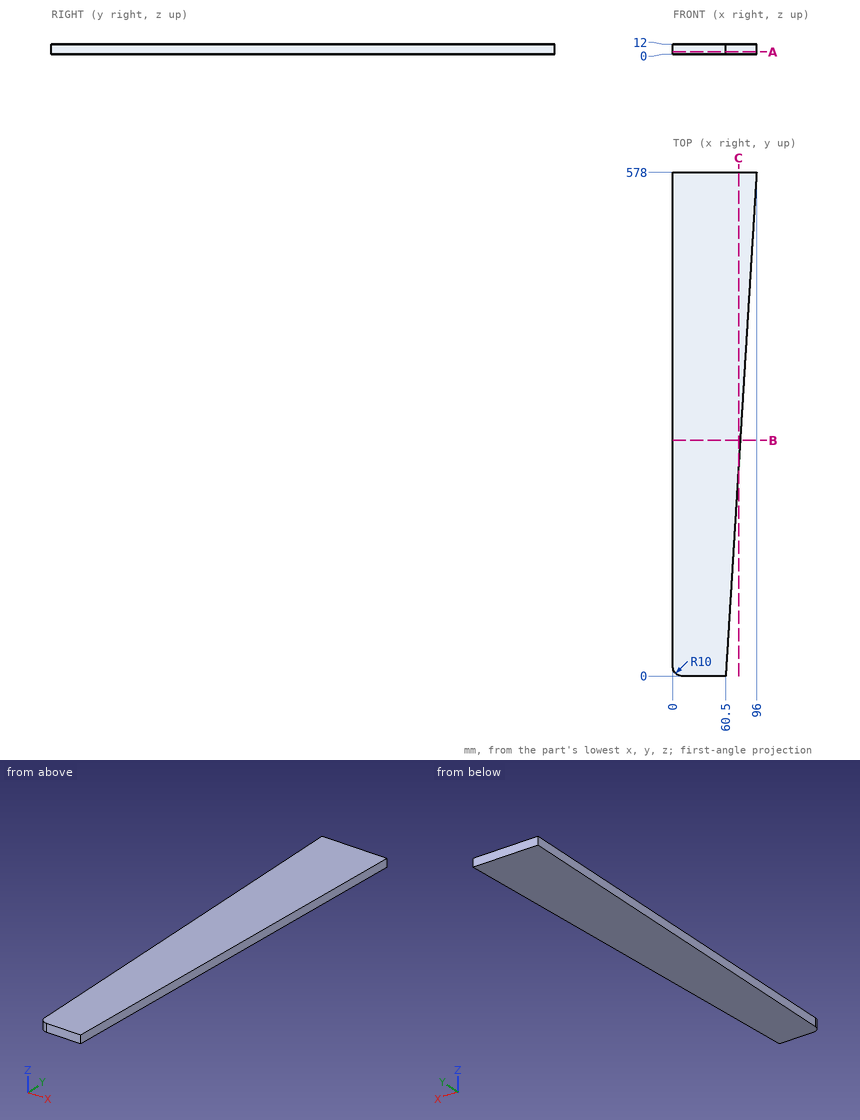
Check sheet for the drawn part. Datum: minimum x, y, z corner. Units: mm. Coordinates: 2 decimals unless noted, no trailing zeros. Loops run counter-clockwise (first coordinate to the right, second up) from the corner with the lowest first, then second, coordinate; pieces in that order, holes last. Notation, with made-up numbers: (30.5, 87) - (59.5, 87) arc R32 ccw to (59.5, 121) - close; hole circle Ø2 at (12.25, -10). An arc over 180 degrees is marked (long way). Put each result on its own line as item: value.
Item 1: Section check C-C (x = 75.5). Enter the section's corners in (y, z).
Conclusion:
outline: (244.23, 0) - (578, 0) - (578, 12) - (244.23, 12) - close
Item 2: Scan lines: line 1 along X through (y, z) = (114, 4.5); line 2 along X through (y, z) = (76, 11). Record each from-to range of solid material in increasing order.
Conclusion:
line 1: x = 0 to 67.5
line 2: x = 0 to 65.17
Item 3: Section check A-A (z = 3). Enter the section's corners in (x, y).
Conclusion:
outline: (0, 10) arc R10 ccw to (10, 0) - (60.5, 0) - (96, 578) - (0, 578) - close
Item 4: Gauge pin test, flat end, axial feed: pin 1 Ø2 at (y, z) = (514.5, 4.5) entering from +X. Record the tip position at first contact, or that the pin passes through.
Conclusion:
pin 1: stops at x = 92.16
Item 5: Section check B-B (y = 270.5). Enter the section's corners in (x, z).
Conclusion:
outline: (0, 0) - (77.11, 0) - (77.11, 12) - (0, 12) - close
